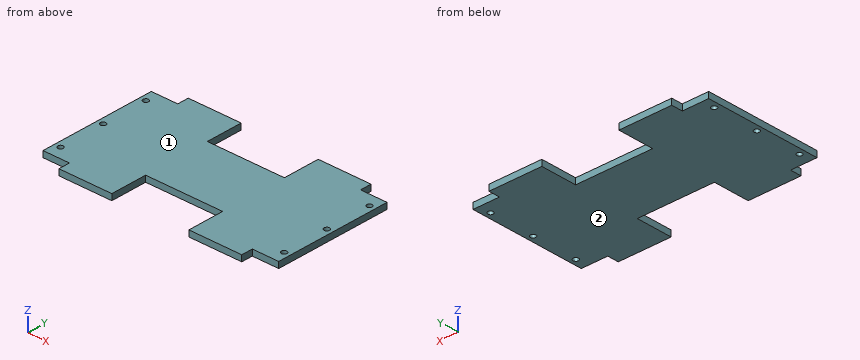
from build123d import *

# Parameters (mm, degrees)
SKETCH1_R           = 18
BOSS_EXTRUDE1_DEPTH = 40


with BuildPart() as part:
    # Sketch1 → Boss-Extrude1 (new body)
    with BuildSketch(Plane.XY):
        Polygon((255, 0), (-255, 0), (-255, -241), (-605, -241), (-605, -166), (-780, -166), (-780, 606), (-605, 606), (-605, 681), (-255, 681), (-255, 440), (255, 440), (255, 681), (605, 681), (605, 606), (780, 606), (780, -166), (605, -166), (605, -241), (255, -241), align=None)
        with Locations((-740, 524)):
            Circle(SKETCH1_R, mode=Mode.SUBTRACT)
        with Locations((-740, 220)):
            Circle(SKETCH1_R, mode=Mode.SUBTRACT)
        with Locations((-740, -84)):
            Circle(SKETCH1_R, mode=Mode.SUBTRACT)
        with Locations(Location((740, 220, 0), (0, 0, 180))):
            Circle(SKETCH1_R, mode=Mode.SUBTRACT)
        with Locations(Location((740, 524, 0), (0, 0, 180))):
            Circle(SKETCH1_R, mode=Mode.SUBTRACT)
        with Locations(Location((740, -84, 0), (0, 0, 180))):
            Circle(SKETCH1_R, mode=Mode.SUBTRACT)
    extrude(amount=BOSS_EXTRUDE1_DEPTH)


solid = part.part
Model file for the job. Use its own axes, mm. Face numbers are marked on the shaded views. Give positions to 0.01 mm unless a question says otherwise; leave off trailing zeros. Loops run counter-clockwise (first coordinate to the right, second up) from the corner with the lowest first, then second, coordinate; pieces in that order, holes last.
Item 1: Drop flat-ended pins along their axis: P1, Ø12, axis at y = 649.5, z = 22, coming from the +X side; P2, Ø12, axis at x = 682.5, z = 14, coming from the +Y side; P3, Ø12, axis at x = 21.5, z = 26.5, coming from the +Y side. Give the stop position or say it passes through.
Check values:
P1: stops at x = 605
P2: stops at y = 606
P3: stops at y = 440
Item 2: Slice it at B-B (z = 27). Write the cut outline in (x, y).
Check values:
outline: (-780, -166) - (-605, -166) - (-605, -241) - (-255, -241) - (-255, 0) - (255, 0) - (255, -241) - (605, -241) - (605, -166) - (780, -166) - (780, 606) - (605, 606) - (605, 681) - (255, 681) - (255, 440) - (-255, 440) - (-255, 681) - (-605, 681) - (-605, 606) - (-780, 606) - close; hole circle Ø36 at (-740, -84); hole circle Ø36 at (-740, 220); hole circle Ø36 at (-740, 524); hole circle Ø36 at (740, -84); hole circle Ø36 at (740, 220); hole circle Ø36 at (740, 524)
Item 3: Drill centre lines: line 1 along Y through (x, z) = (-740, 30.5); line 2 along X through (y, z) = (-128.5, 4.5); line 3 along Y through (x, z) = (-68.5, 37.5). Where is each one in solid material? Low to high.
Check values:
line 1: y = -166 to -102, -66 to 202, 238 to 506, 542 to 606
line 2: x = -780 to -255, 255 to 780
line 3: y = 0 to 440
Item 4: Mould opens along Z. For the marked faces 1 and 2 say: +Z half, -Z half, draft (parallel to the pull), parting line (faces both ways), or undercut.
Check values:
face 1: +Z half
face 2: -Z half
Item 5: Slice it at C-C (x = -740). Write the cut outline in (y, z), plus the area to 3 significant figures.
Check values:
outline: (-166, 0) - (-102, 0) - (-102, 40) - (-166, 40) - close; (-66, 0) - (202, 0) - (202, 40) - (-66, 40) - close; (238, 0) - (506, 0) - (506, 40) - (238, 40) - close; (542, 0) - (606, 0) - (606, 40) - (542, 40) - close
area: 26,600 mm2
Item 6: Slice it at D-D (y = 220). Write the cut outline in (x, z).
Check values:
outline: (-780, 0) - (-758, 0) - (-758, 40) - (-780, 40) - close; (-722, 0) - (722, 0) - (722, 40) - (-722, 40) - close; (758, 0) - (780, 0) - (780, 40) - (758, 40) - close
Item 7: Slice it at A-A (y = -183). Write the cut outline in (x, z).
Check values:
outline: (-605, 0) - (-255, 0) - (-255, 40) - (-605, 40) - close; (255, 0) - (605, 0) - (605, 40) - (255, 40) - close
